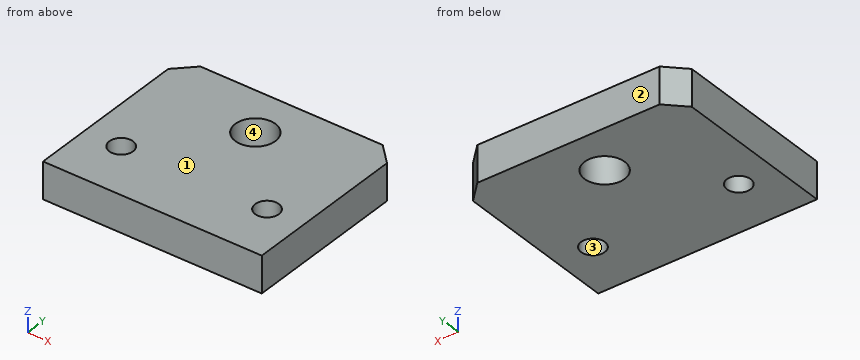
from build123d import *

# Parameters (mm, degrees)
SKETCH1_W           = 60
SKETCH1_H           = 50
BOSS_EXTRUDE1_DEPTH = 10
SKETCH2_R           = 5.5
CUT_EXTRUDE1_DEPTH  = 18
CHAMFER1_SIZE       = 5
SKETCH3_R           = 3.25
CUT_EXTRUDE2_DEPTH  = 46.967787324


with BuildPart() as part:
    # Sketch1 → Boss-Extrude1 (new body)
    with BuildSketch(Plane.XY):
        with Locations((-5.243851729, -2.76523702)):
            Rectangle(SKETCH1_W, SKETCH1_H)
    extrude(amount=BOSS_EXTRUDE1_DEPTH)

    # Sketch2 → Cut-Extrude1 (cut)
    with BuildSketch(Plane(origin=(0, 0, 0), x_dir=(-1, 0, 0), z_dir=(0, 0, -1))):
        with Locations((5.243851729, 9.23476298)):
            Circle(SKETCH2_R)
    extrude(amount=-CUT_EXTRUDE1_DEPTH, mode=Mode.SUBTRACT)

    # Chamfer1
    chamfer1_edges = [part.edges().sort_by_distance(p)[0] for p in [
        (-35.243851729, 22.23476298, 5),
        (24.756148271, 22.23476298, 5),
    ]]
    chamfer(chamfer1_edges, length=CHAMFER1_SIZE)

    # Sketch3 → Cut-Extrude2 (cut, through all)
    with BuildSketch(Plane(origin=(0, 0, 0), x_dir=(-1, 0, 0), z_dir=(0, 0, -1))):
        with Locations((-14.756148271, -12.76523702)):
            Circle(SKETCH3_R)
        with Locations((25.243851729, -12.76523702)):
            Circle(SKETCH3_R)
    extrude(amount=-CUT_EXTRUDE2_DEPTH, mode=Mode.SUBTRACT)


solid = part.part
Model file for the job. Use its own axes, mm. Face numbers are marked on the shaded views. Round coordinates to 2 decimals unless told otherwise and drop trailing zeros. Loops run counter-clockwise (first coordinate to the right, second up) from the corner with the lowest first, then second, coordinate; pieces in that order, holes last. Notation, with made-up numbers: (61, 2.5) - (72, 2.5) arc R29 cw to (72, 25.5) - close; hole circle Ø9 at (23, -17). An arc over 180 degrees is marked (long way). Write each question's results on one line, items separated by ' | '.
(1) Saw through at A-A, the plane x = -1. List the corners of the cut face in (y, z).
Answer below:
outline: (-27.77, 0) - (5.74, 0) - (5.74, 10) - (-27.77, 10) - close; (12.73, 0) - (22.23, 0) - (22.23, 10) - (12.73, 10) - close
(2) Saw through at B-B, the plane z = 5.5. List the corners of the cut face in (x, y), then the cut area to 3 significant figures.
Answer below:
outline: (-35.24, -27.77) - (24.76, -27.77) - (24.76, 17.23) - (19.76, 22.23) - (-30.24, 22.23) - (-35.24, 17.23) - close; hole circle Ø6.5 at (-25.24, -12.77); hole circle Ø11 at (-5.24, 9.23); hole circle Ø6.5 at (14.76, -12.77) | area: 2,810 mm^2
(3) Mould opens along Y. For the marked faces 1, 2, 3 and 4 say: released by +Y, released by -Y, zero draft, split by the parting line, or undercut.
Answer below:
face 1: zero draft | face 2: released by +Y | face 3: undercut | face 4: undercut
(4) Wall check: L1, parallel to Y at x = 14.5, z = 8; L2, parallel to X at y = 11, z = 0.5; L3, parallel to X at y = 5.5, z = 3. Give the ranges that are in metal, low to high.
Answer below:
L1: y = -27.77 to -16.01, -9.53 to 22.23 | L2: x = -35.24 to -10.45, -0.03 to 24.76 | L3: x = -35.24 to -9.28, -1.21 to 24.76
